Verification items for the finished model (mm, model axes). A direction names the side the tool comes from. Round coordinates to 2 decimals unless told otherwise and drop trailing zeros. Write each loop counter-clockwise with the first axis right and the second up, starting at its lowest first coordinate (ties: lowest second). Pieces come first, ordered by that corner, then holes.
from build123d import *

# Parameters (mm, degrees)
GB_6728_1986_050_X_50_X_3_1_DEPTH = 670


with BuildPart() as part:
    # Sketch1 → Gb／6728-1986方形空心型钢 050 X 50 X 3(1) (new body)
    with BuildSketch(Plane.YX.offset(-335)):
        with BuildLine():
            Line((-19, -25), (19, -25))
            ThreePointArc((19, -25), (23.242640687, -23.242640687), (25, -19))
            Line((25, -19), (25, 19))
            ThreePointArc((25, 19), (23.242640687, 23.242640687), (19, 25))
            Line((19, 25), (-19, 25))
            ThreePointArc((-19, 25), (-23.242640687, 23.242640687), (-25, 19))
            Line((-25, 19), (-25, -19))
            ThreePointArc((-25, -19), (-23.242640687, -23.242640687), (-19, -25))
        make_face()
        with BuildLine():
            Line((-19, -22), (19, -22))
            ThreePointArc((19, -22), (21.121320344, -21.121320344), (22, -19))
            Line((22, -19), (22, 19))
            ThreePointArc((22, 19), (21.121320344, 21.121320344), (19, 22))
            Line((19, 22), (-19, 22))
            ThreePointArc((-19, 22), (-21.121320344, 21.121320344), (-22, 19))
            Line((-22, 19), (-22, -19))
            ThreePointArc((-22, -19), (-21.121320344, -21.121320344), (-19, -22))
        make_face(mode=Mode.SUBTRACT)
    extrude(amount=GB_6728_1986_050_X_50_X_3_1_DEPTH)


solid = part.part
Q1. Sectioned sample at A-A (y = 4.5). Enter the section's corners in (x, z), plus the area to 3 significant figures.
Recorded:
outline: (-25, -335) - (-22, -335) - (-22, 335) - (-25, 335) - close; (22, -335) - (25, -335) - (25, 335) - (22, 335) - close
area: 4,020 mm2
Q2. Tool access check on faces 1 (the flat face through (25, 0, 5)), 2 (the flat face through (22, 0, 5)). Record the directions out of +Z, -Z, +X, -X, +Y, -Y that give a thin tool (end or side, any length) a straight path to the whole face; none if there is none.
Recorded:
face 1: +Z, -Z, +X, +Y, -Y
face 2: +Z, -Z
Q3. Release check for a two-part mould opening along Y. For faces 3 (the flat face through (0.1, -22.3, -335)), 4 (the flat face through (-22, 0, 5)), 5 (the flat face through (0, 25, 5)) record: released by +Y, released by -Y, zero draft, split by the parting line, or undercut.
Recorded:
face 3: zero draft
face 4: undercut
face 5: released by +Y
Q4. Material ranges on line 1 along X through (y, z) = (-17.5, 67.5); line 2 along Y through (x, z) = (21.5, -140.5), recorded low to high.
Recorded:
line 1: x = -25 to -22, 22 to 25
line 2: y = -24.45 to -20.66, 20.66 to 24.45
Q5. Sectioned sample at C-C (z = 62). Enter the section's corners in (x, y), plus the area to 3 significant figures.
Recorded:
outline: (-25, -19) arc R6 ccw to (-19, -25) - (19, -25) arc R6 ccw to (25, -19) - (25, 19) arc R6 ccw to (19, 25) - (-19, 25) arc R6 ccw to (-25, 19) - close; hole (-22, -19) arc R3 ccw to (-19, -22) - (19, -22) arc R3 ccw to (22, -19) - (22, 19) arc R3 ccw to (19, 22) - (-19, 22) arc R3 ccw to (-22, 19) - close
area: 541 mm2
